Part model, mm, in its own coordinate system. Give positions to 0.01 mm unless a question says otherwise; leave off trailing zeros. Order: outer loops, then holes, each group sorted by start corner. A loop starts at its lowest first (then second) coordinate and runs counter-clockwise, first axis right, second up. Notation, with made-up numbers: M 16.25,16.25 L 25.25,16.25 A35 cw 25.25,53.25 Z; hole C 48.5,-29.75 d8. An arc over 180 degrees is marked long. Answer as a JSON object with one key per item and string values.
from build123d import *

# Parameters (mm, degrees)
SKETCH1_R           = 2.1
BOSS_EXTRUDE1_DEPTH = 5


with BuildPart() as part:
    # Sketch1 → Boss-Extrude1 (new body)
    with BuildSketch(Plane.XY):
        Polygon((30, 300), (30, 220), (35, 220), (35, 145), (30, 145), (30, 80), (35, 80), (35, 0), (0, 0), (0, 300), align=None)
        with Locations((25, 215)):
            Circle(SKETCH1_R, mode=Mode.SUBTRACT)
        with Locations((10, 215)):
            Circle(SKETCH1_R, mode=Mode.SUBTRACT)
        with Locations((25, 75)):
            Circle(SKETCH1_R, mode=Mode.SUBTRACT)
        with Locations((10, 75)):
            Circle(SKETCH1_R, mode=Mode.SUBTRACT)
        with Locations((10, 290)):
            Circle(SKETCH1_R, mode=Mode.SUBTRACT)
        with Locations((10, 10)):
            Circle(SKETCH1_R, mode=Mode.SUBTRACT)
        with Locations((25, 30)):
            Circle(SKETCH1_R, mode=Mode.SUBTRACT)
        with Locations((25, 50)):
            Circle(SKETCH1_R, mode=Mode.SUBTRACT)
    extrude(amount=BOSS_EXTRUDE1_DEPTH)


solid = part.part
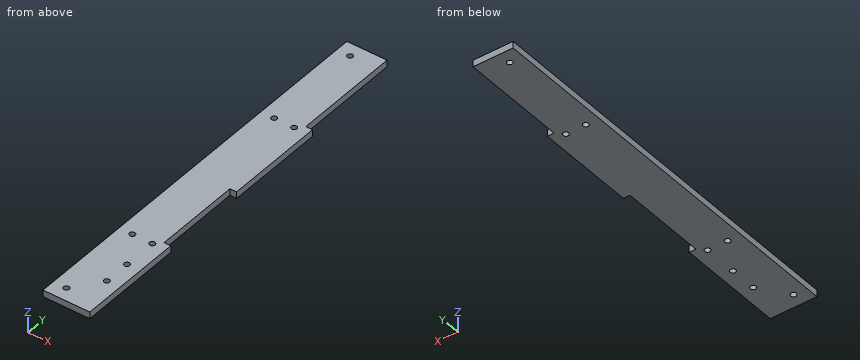
1. Pin check, flat tips, straight feed: P1, Ø3.5, axis at x = 10, y = 75, coming from the -Z side; P2, Ø2.5, axis at y = 246.5, z = 2.5, coming from the +X side; P3, Ø2.5, axis at x = 33.5, z = 3.5, coming from the +Y side. Stop position of each tip, or through.
Worked answers:
{"P1": "passes through", "P2": "stops at x = 30", "P3": "stops at y = 220"}
2. Cut at B-B on y = 265. Give the cut face in (x, z), plus the area to 3 significant figures.
Worked answers:
{"outline": "M 0,0 L 30,0 L 30,5 L 0,5 Z", "area": "150 mm^2"}
3. Cut at A-A on z = 3.45. State how many separate pieces and enclosed holes the cut face has, plus the area to 3 significant figures.
Worked answers:
{"separate pieces": "1", "enclosed holes": "8", "area": "9,660 mm^2"}
4. Probe line 1 along Y through (x, z) = (10, 1.8); line 2 along Y through (x, z) = (25, 1.95); line 3 along X through (y, z) = (215.5, 2). List the from-to ranges inside material, lowest first.
Worked answers:
{"line 1": "y = 0 to 7.9, 12.1 to 72.9, 77.1 to 212.9, 217.1 to 287.9, 292.1 to 300", "line 2": "y = 0 to 27.9, 32.1 to 47.9, 52.1 to 72.9, 77.1 to 212.9, 217.1 to 300", "line 3": "x = 0 to 7.96, 12.04 to 22.96, 27.04 to 35"}
